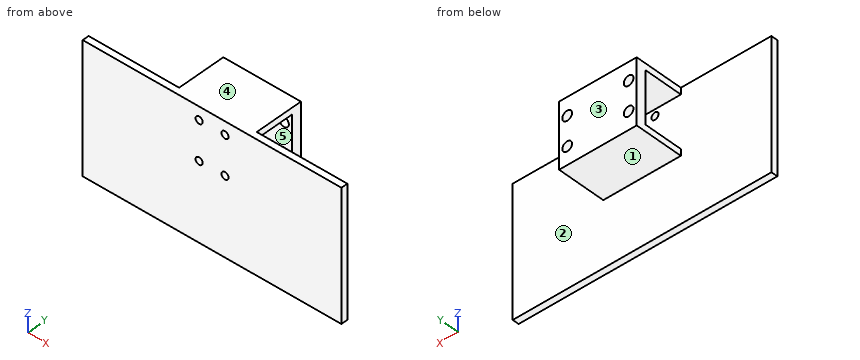
from build123d import *

# Parameters (mm, degrees)
SKETCH1_W           = 80
SKETCH1_H           = 20
SKETCH1_R           = 1.1
BOSS_EXTRUDE1_DEPTH = 2
BOSS_EXTRUDE3_DEPTH = 12
SKETCH4_R           = 1.5
CUT_EXTRUDE1_DEPTH  = 5
SKETCH5_W           = 80
SKETCH5_H           = 2
BOSS_EXTRUDE4_DEPTH = 20


with BuildPart() as part:
    # Sketch1 → Boss-Extrude1 (new body)
    with BuildSketch(Plane(origin=(0, 0, 0), x_dir=(1, 0, 0), z_dir=(0, 1, 0))):
        Rectangle(SKETCH1_W, SKETCH1_H)
        with Locations(Location((-4, 6, 0), (0, 0, 270))):
            Circle(SKETCH1_R, mode=Mode.SUBTRACT)
        with Locations(Location((4, 6, 0), (0, 0, 270))):
            Circle(SKETCH1_R, mode=Mode.SUBTRACT)
        with Locations(Location((-4, -6, 0), (0, 0, 270))):
            Circle(SKETCH1_R, mode=Mode.SUBTRACT)
        with Locations(Location((4, -6, 0), (0, 0, 270))):
            Circle(SKETCH1_R, mode=Mode.SUBTRACT)
    extrude(amount=BOSS_EXTRUDE1_DEPTH)

    # Sketch3 → Boss-Extrude3 (add, symmetric)
    with BuildSketch(Plane(origin=(0, 0, 0), x_dir=(0, 0, -1), z_dir=(1, 0, 0))):
        Polygon((-10, 2), (-8, 2), (-8, 14), (8, 14), (8, 2), (10, 2), (10, 13.782871327), (10, 17), (-10, 17), (-10, 13.782871327), align=None)
    extrude(amount=BOSS_EXTRUDE3_DEPTH, both=True)

    # Sketch4 → Cut-Extrude1 (cut)
    with BuildSketch(Plane(origin=(0, 17, 0), x_dir=(1, 0, 0), z_dir=(0, 1, 0))):
        with Locations(Location((9.5, -4.5, 0), (0, 0, 270))):
            Circle(SKETCH4_R)
        with Locations(Location((-9.5, -4.5, 0), (0, 0, 270))):
            Circle(SKETCH4_R)
        with Locations(Location((-9.5, 4.5, 0), (0, 0, 270))):
            Circle(SKETCH4_R)
        with Locations(Location((9.5, 4.5, 0), (0, 0, 270))):
            Circle(SKETCH4_R)
    extrude(amount=-CUT_EXTRUDE1_DEPTH, mode=Mode.SUBTRACT)

    # Sketch5 → Boss-Extrude4 (add)
    with BuildSketch(Plane.XY.offset(-10)):
        with Locations((0, 1)):
            Rectangle(SKETCH5_W, SKETCH5_H)
    extrude(amount=-BOSS_EXTRUDE4_DEPTH)


solid = part.part
Model file for the job. Use its own axes, mm. Face numbers are marked on the shaded views. A direction names the side the tool comes from. Round coordinates to 2 decimals unless told otherwise and drop trailing zeros. Order: outer loops, then holes, each group sorted by start corner. A loop starts at its lowest first (then second) coordinate and runs counter-clockwise, first axis right, second up. Notation, with made-up numbers: M 81,74.5 L 109,74.5 A31 cw 109,104.5 Z; hole C 2.5,-17.75 d9. An arc over 180 degrees is marked long. Write each question's results on one line, items separated by ' | '. Start each with the question number.
(1) Which spindle directions (+Z, -Z, +X, -X, +Y, -Y) get a long thin tool onto all of the face, cutting with end or side? Do the marked faces 4 and 5. Say none if no direction does.
(2) Probe probe 1 along X at (y, z) = (0.9, 6); probe 2 along X at (y, z) = (15.8, 4.5); probe 3 along Z at (x, y) = (-11.5, 5.75). List the from-to ranges inside material, lowest first. Write a range as from..to.
(3) Saw through at C-C, the plane x = 1. Give the cut face in (y, z), then the cut area to 3 significant figures.
(4) Saw through at D-D, the plane z = -4. Give the cut face in (x, y).
(5) Two-plate mould, pull along Z, no slides. Class the marked faces 1, 2 and 3: pulls with the +Z half, pulls with the -Z half, needs draft (parallel to the pull), parting line crosses it, or undercut.
(6) Drop flat-ended pins along their axis: pin 1 (2.5 mm diameter, centred on x = 9.5, z = 4.5, fed in from +Y); pin 2 (7.5 mm diameter, centred on y = 13, z = 1, fed in from -X). Give the stop position or say it passes through.
(7) Saw through at B-B, the plane y = 5. Give the cut face in (x, z).
(8) Saw through at A-A, the plane x = 9.5. Give the cut face in (y, z), then the cut area to 3 significant figures.
Established:
1) face 4: +Z, +X, -X, +Y, -Y | face 5: +X, -X
2) probe 1: x = -40..-5.1, -2.9..2.9, 5.1..40 | probe 2: x = -12..-11, -8..8, 11..12 | probe 3: z = -10..-8, 8..10
3) outline: M 0,-30 L 2,-30 L 2,-10 L 17,-10 L 17,10 L 0,10 Z; hole M 2,-8 L 14,-8 L 14,8 L 2,8 Z | area: 188 mm^2
4) outline: M -40,0 L 40,0 L 40,2 L -40,2 Z; M -12,14 L -10.91,14 L -10.91,17 L -12,17 Z; M -8.09,14 L 8.09,14 L 8.09,17 L -8.09,17 Z; M 10.91,14 L 12,14 L 12,17 L 10.91,17 Z
5) face 1: pulls with the -Z half | face 2: undercut | face 3: needs draft
6) pin 1: stops at y = 2 | pin 2: stops at x = -12
7) outline: M -12,-10 L 12,-10 L 12,-8 L -12,-8 Z; M -12,8 L 12,8 L 12,10 L -12,10 Z
8) outline: M 0,-30 L 2,-30 L 2,-10 L 17,-10 L 17,-6 L 14,-6 L 14,-8 L 2,-8 L 2,8 L 14,8 L 14,6 L 17,6 L 17,10 L 0,10 Z; M 14,-3 L 17,-3 L 17,3 L 14,3 Z | area: 170 mm^2
